Print and shaded views of the part. All mm, measured from the part's lowest x, y and z. A direction names the side the tool comes from. Give positions to 0.01 mm unless a question says otherwise; leave off trailing zeros. Order: outer loops, then holes, each group sorted by start corner. A loop starts at its lowest first (then second) coordinate and runs counter-clockwise, first axis right, second up. Notation, with made-up numbers: (-20.5, -13.75) - (34.5, -13.75) arc R9 cw to (34.5, 0.25) - close; hole circle Ø3 at (73, 29.25). An arc over 180 degrees is marked (long way). Answer in a Markdown table with one row per item.
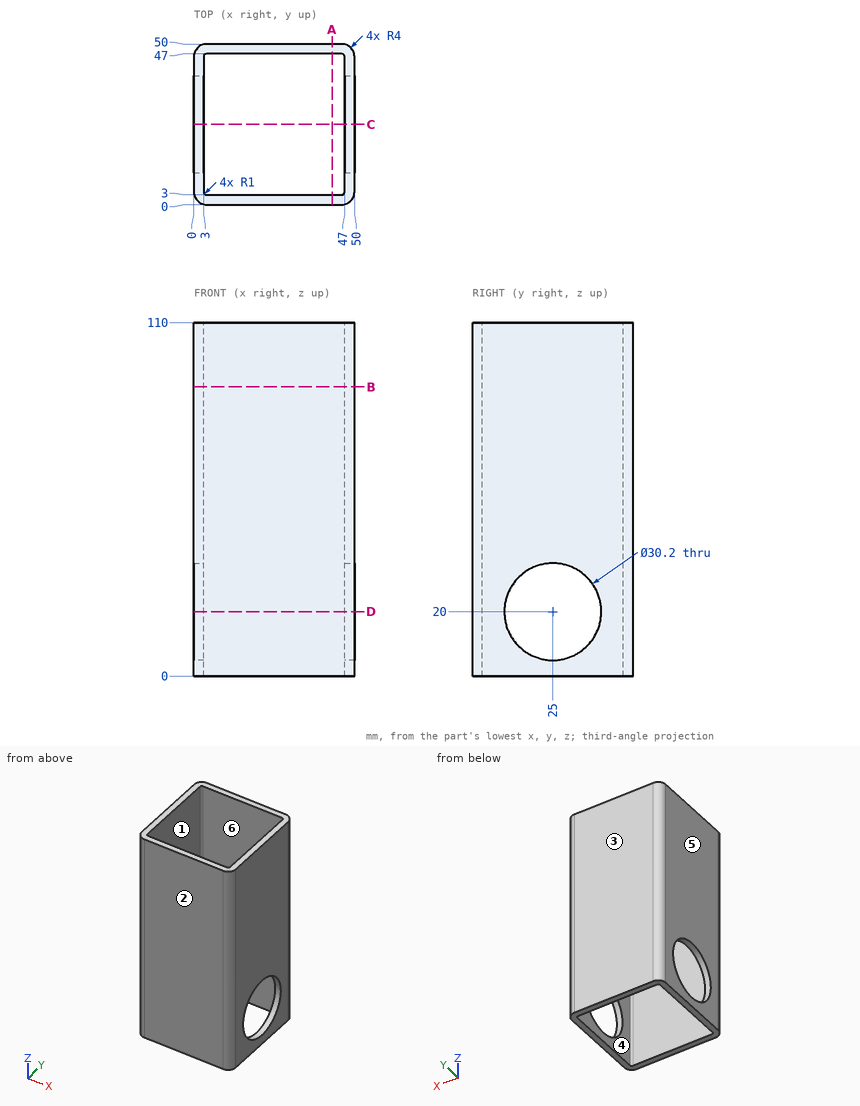
1. Cut at C-C on y = 25. Write the cut outline in (x, z).
Check result:
| item | result |
|---|---|
| outline | (0, 0) - (3, 0) - (3, 4.9) - (0, 4.9) - close; (0, 35.1) - (3, 35.1) - (3, 110) - (0, 110) - close; (47, 0) - (50, 0) - (50, 4.9) - (47, 4.9) - close; (47, 35.1) - (50, 35.1) - (50, 110) - (47, 110) - close |
2. Which spindle directions (+Z, -Z, +X, -X, +Y, -Y) get a long thin tool onto all of the face, cutting with end or side? Do the marked faces 1 and 2. Say none if no direction does.
Check result:
| item | result |
|---|---|
| face 1 | +Z, -Z |
| face 2 | +Z, -Z, +X, -X, -Y |
3. Probe line 1 (X direction, y = 9.5, z = 26.5); line 2 (Y direction, x = 48.2, z = 20). List the from-to ranges inside material, lowest first.
Check result:
| item | result |
|---|---|
| line 1 | x = 0 to 3, 47 to 50 |
| line 2 | y = 0.66 to 9.9, 40.1 to 49.34 |
4. Cut at D-D on z = 20. Write the cut outline in (x, y).
Check result:
| item | result |
|---|---|
| outline | (0, 4) arc R4 ccw to (4, 0) - (46, 0) arc R4 ccw to (50, 4) - (50, 9.9) - (47, 9.9) - (47, 4) arc R1 cw to (46, 3) - (4, 3) arc R1 cw to (3, 4) - (3, 9.9) - (0, 9.9) - close; (0, 40.1) - (3, 40.1) - (3, 46) arc R1 cw to (4, 47) - (46, 47) arc R1 cw to (47, 46) - (47, 40.1) - (50, 40.1) - (50, 46) arc R4 ccw to (46, 50) - (4, 50) arc R4 ccw to (0, 46) - close |
5. Two-plate mould, pull along Y, no slides. Class the marked faces 3, 4, 5 and 6: +Y half, -Y half, draft (parallel to the pull), parting line (faces both ways), or undercut.
Check result:
| item | result |
|---|---|
| face 3 | +Y half |
| face 4 | undercut |
| face 5 | draft |
| face 6 | undercut |
6. Cut at A-A on x = 43. Write the cut outline in (y, z), and give its area (3 significant figures).
Check result:
| item | result |
|---|---|
| outline | (0, 0) - (3, 0) - (3, 110) - (0, 110) - close; (47, 0) - (50, 0) - (50, 110) - (47, 110) - close |
| area | 660 mm² |
7. Cut at B-B on z = 90. Write the cut outline in (x, y), and give its area (3 significant figures).
Check result:
| item | result |
|---|---|
| outline | (0, 4) arc R4 ccw to (4, 0) - (46, 0) arc R4 ccw to (50, 4) - (50, 46) arc R4 ccw to (46, 50) - (4, 50) arc R4 ccw to (0, 46) - close; hole (3, 4) arc R1 ccw to (4, 3) - (46, 3) arc R1 ccw to (47, 4) - (47, 46) arc R1 ccw to (46, 47) - (4, 47) arc R1 ccw to (3, 46) - close |
| area | 551 mm² |
8. Drop a flat-ended pin along its axis: P1, Ø2, axis at x = 14, z = 24.5, coming from the -Y side. Give the stop position or say it passes through.
Check result:
| item | result |
|---|---|
| P1 | stops at y = 0 |
